```python
from build123d import *

# Parameters (mm, degrees)
BOSS_EXTRUDE1_DEPTH   = 15
M8_TAPPED_HOLE1_D     = 6.8
M8_TAPPED_HOLE1_DEPTH = 22.25
M8_TAPPED_HOLE1_TIP   = 2.042926105
M8_TAPPED_HOLE2_D     = 6.8
M8_TAPPED_HOLE2_DEPTH = 22.25
M8_TAPPED_HOLE2_TIP   = 2.042926105


with BuildPart() as part:
    # Sketch1 → Boss-Extrude1 (new body)
    with BuildSketch(Plane.XY):
        Polygon((0, 0), (0, 50), (80, 50), (80, 45), (5, 0), align=None)
    extrude(amount=BOSS_EXTRUDE1_DEPTH)

    # M8 Tapped Hole1
    with Locations(Plane(origin=(0, 50, 0), x_dir=(1, 0, 0), z_dir=(0, 1, 0))):
        with Locations((25, -7.5), (50, -7.5)):
            Hole(M8_TAPPED_HOLE1_D / 2, depth=M8_TAPPED_HOLE1_DEPTH)
            with Locations((0, 0, -(M8_TAPPED_HOLE1_DEPTH + M8_TAPPED_HOLE1_TIP / 2))):  # 118° drill point
                Cone(0, M8_TAPPED_HOLE1_D / 2, M8_TAPPED_HOLE1_TIP, mode=Mode.SUBTRACT)

    # M8 Tapped Hole2
    with Locations(Plane.ZY):
        with Locations((7.5, 35), (7.5, 15)):
            Hole(M8_TAPPED_HOLE2_D / 2, depth=M8_TAPPED_HOLE2_DEPTH)
            with Locations((0, 0, -(M8_TAPPED_HOLE2_DEPTH + M8_TAPPED_HOLE2_TIP / 2))):  # 118° drill point
                Cone(0, M8_TAPPED_HOLE2_D / 2, M8_TAPPED_HOLE2_TIP, mode=Mode.SUBTRACT)


solid = part.part
```
Could you check a few things on this model? Use its own coordinates, in mm. A direction names the side the tool comes from. Coordinates: 2 decimals unless noted, no trailing zeros. Write each loop counter-clockwise with the first axis right and the second up, starting at its lowest first coordinate (ties: lowest second). Pieces come first, ordered by that corner, then holes. Notation, with made-up numbers: (64.5, 52.5) -> (108.5, 52.5) arc R21 ccw to (108.5, 56.5) -> close; hole circle Ø10 at (60, -12). An arc over 180 degrees is marked (long way). Return JSON: item names as keys, results as strings.
(1) Imagine slicing it at C-C, the plane x = 50. Please give me the cut outline in (y, z).
Numbers:
{"outline": "(27, 0) -> (50, 0) -> (50, 4.1) -> (27.75, 4.1) -> (27, 5.35) -> close; (27, 9.65) -> (27.75, 10.9) -> (50, 10.9) -> (50, 15) -> (27, 15) -> close"}
(2) We'd pull the mould along Y, two halves only. Please class faces 1 (the flat face through (43, 22.8, 7.4)), 2 (the cylindrical face through (28.4, 38.7, 7.4)), 3 (the conical face through (23.938, 15.498, 7.817)): +Y half, -Y half, draft (parallel to the pull), parting line (faces both ways), or undercut.
Numbers:
{"face 1": "-Y half", "face 2": "draft", "face 3": "undercut"}
(3) I'm going to push flat-ended pins straight in: pin 1 (9 mm diameter, centred on y = 15, z = 7.5, fed in from +X); pin 2 (5 mm diameter, centred on y = 32, z = 2, fed in from +X); pin 3 (4 mm diameter, centred on y = 35, z = 7.5, fed in from +X). Where does each tip first touch, or does it pass through?
Numbers:
{"pin 1": "stops at x = 37.5", "pin 2": "stops at x = 62.5", "pin 3": "stops at x = 66.67"}
(4) Which directions (+Z, -Z, +X, -X, +Y, -Y) give clear straight access to the entire face, cutting with the end or side of a thin tool? Please do faces 4 (the cylindrical face through (46.86, 38.72, 8.8)), 5 (the cylindrical face through (11.281, 37.867, 5.672)), 6 (the flat face through (80, 48, 7)).
Numbers:
{"face 4": "+Y", "face 5": "-X", "face 6": "+Z, -Z, +X, +Y, -Y"}
(5) Imagine slicing it at B-B, the plane z = 12.25. Please give me the cut outline in (x, y).
Numbers:
{"outline": "(0, 0) -> (5, 0) -> (80, 45) -> (80, 50) -> (0, 50) -> close"}
(6) Imagine slicing it at D-D, the plane x = 32. Please give me the cut outline in (y, z).
Numbers:
{"outline": "(16.2, 0) -> (50, 0) -> (50, 15) -> (16.2, 15) -> close"}
(7) I need wall thicknesses on L1, parallel to Z at x = 12.25, y = 35; L2, parallel to Y at x = 5, z = 6.75; L3, parallel to Y at x = 4, z = 10.5. Which ranges of each line are inside material? Lowest first, please.
Numbers:
{"L1": "z = 0 to 4.1, 10.9 to 15", "L2": "y = 0 to 11.68, 18.32 to 31.68, 38.32 to 50", "L3": "y = 0 to 13.4, 16.6 to 33.4, 36.6 to 50"}
(8) Imagine slicing it at A-A, the plane y = 35. Please give me the cut outline in (x, z).
Numbers:
{"outline": "(0, 0) -> (63.33, 0) -> (63.33, 15) -> (0, 15) -> (0, 10.9) -> (22.25, 10.9) -> (22.76, 10.06) arc R3.4 cw (long way) to (22.76, 4.94) -> (22.25, 4.1) -> (0, 4.1) -> close; hole circle Ø6.8 at (50, 7.5)"}
